from build123d import *

# Parameters (mm, degrees)
EXTRUDE_START          = 700
SKETCH_1_R             = 15
EXTRUDE_1_DEPTH        = 15
PATTERN_LINEAR_1_COUNT = 2
PATTERN_LINEAR_1_PITCH = 77
SKETCH_2_W             = 62
SKETCH_2_H             = 7
EXTRUDE_2_DEPTH        = 70
SKETCH_3_R             = 11
CUT_EXTRUDE_2_DEPTH    = 105
FILLET_1_R             = 5


with BuildPart() as part:
    # Sketch 1 → Extrude 1 (new body)
    with BuildSketch(Plane.XY.offset(-2290.827909759).offset(EXTRUDE_START)):
        with BuildLine():
            Line((4, 81), (-196, 81))
            ThreePointArc((-196, 81), (-230.605231181, 110.758056189), (-206.365638709, 149.429830005))
            Line((-206.365638709, 149.429830005), (-111, 179))
            Line((-111, 179), (17.209362926, 179))
            ThreePointArc((17.209362926, 179), (40.340952707, 173.32752592), (58.22400875, 157.597182169))
            Line((58.22400875, 157.597182169), (67.202929165, 144.719436434))
            ThreePointArc((67.202929165, 144.719436434), (67.865505184, 134.373682044), (59, 129))
            Line((59, 129), (4, 129))
            Line((4, 129), (4, 81))
        make_face()
        with Locations((-196, 116)):
            Circle(SKETCH_1_R, mode=Mode.SUBTRACT)
    extrude(amount=EXTRUDE_1_DEPTH)


with BuildPart() as pattern_linear_1_1:
    # Pattern Linear 1: pattern copy
    add(part.part.moved(Location(Vector(0, 0, 1) * (1 * PATTERN_LINEAR_1_PITCH))))


with BuildPart() as part_1:
    add(part.part)

    add(pattern_linear_1_1.part)  # Extrude 2 merges Pattern Linear 1_1
    # Sketch 2 → Extrude 2 (add)
    with BuildSketch(Plane.ZY.offset(-4)):
        with Locations((-1544.827909759, 120.5)):
            Rectangle(SKETCH_2_W, SKETCH_2_H)
    extrude(amount=EXTRUDE_2_DEPTH)

    # Sketch 3 → Cut-Extrude 2 (cut, symmetric)
    with BuildSketch(Plane(origin=(0, 0, -1513.827909759), x_dir=(-1, 0, 0), z_dir=(0, 0, -1))):
        with Locations(Location((80.605231181, 144, 0), (0, 0, 180))):
            Circle(SKETCH_3_R)
    extrude(amount=CUT_EXTRUDE_2_DEPTH, both=True, mode=Mode.SUBTRACT)

    # Fillet 1
    fillet_1_edges = [part_1.edges().sort_by_distance(p)[0] for p in [
        (4, 129, -1583.327909759),
        (4, 129, -1506.327909759),
    ]]
    fillet(fillet_1_edges, radius=FILLET_1_R)


solid = part_1.part
Can you work these out from the model? Positions are in its coordinate system, mm. A direction names the side the tool comes from. Coordinates: 2 decimals unless noted, no trailing zeros. Write each loop counter-clockwise with the first axis right and the second up, starting at its lowest first coordinate (ties: lowest second). Pieces come first, ordered by that corner, then holes.
Q1. Which directions (+Z, -Z, +X, -X, +Y, -Y) give clear straight access to the entire face, cutting with the end or side of a thin tool? Please do faces 4 (the face through (-31, 124, -1545)), 5 (the face through (-66, 121, -1545)), 6 (the face through (62.65, 151.25, -1583.43)), 7 (the face through (-31, 117, -1545)), 8 (the face through (34, 129, -1583)).
Results found:
face 4: +X, -X, +Y
face 5: -X, +Y, -Y
face 6: +Z, -Z, +X, +Y
face 7: +X, -X, -Y
face 8: +Z, -Z, +X, -Y
Q2. Imagine slicing it at B-B, the plane x = -6.5. List the corners of the cut face in (y, z) for me.
Results found:
outline: (81, -1590.83) - (179, -1590.83) - (179, -1575.83) - (124, -1575.83) - (124, -1513.83) - (179, -1513.83) - (179, -1498.83) - (81, -1498.83) - (81, -1513.83) - (117, -1513.83) - (117, -1575.83) - (81, -1575.83) - close
Q3. Imagine slicing it at D-D, the plane y = 90.5. List the corners of the cut face in (x, z) for me, plus the area to 3 significant figures.
Results found:
outline: (-219.97, -1590.83) - (4, -1590.83) - (4, -1575.83) - (-219.97, -1575.83) - close; (-219.97, -1513.83) - (4, -1513.83) - (4, -1498.83) - (-219.97, -1498.83) - close
area: 6,720 mm2
Q4. Imagine slicing it at C-C, the plane x = -137.5. List the corners of the cut face in (y, z) for me, plus the area to 3 significant figures.
Results found:
outline: (81, -1590.83) - (170.78, -1590.83) - (170.78, -1575.83) - (81, -1575.83) - close; (81, -1513.83) - (170.78, -1513.83) - (170.78, -1498.83) - (81, -1498.83) - close
area: 2,690 mm2
Q5. For P1, Ø7.5, axis at y = 120, z = -1554, coming from the -X side; P2, Ø4, axis at x = -71.5, z = -1517.5, coming from the +Y side; P3, Ø6, axis at x = -68.5, z = -1530, coming from the +Y side; P4, Ø7.5, axis at x = 38, z = -1584.5, coming from the -Y side, each with a flat end and sliding along its axis, tell me the tip position at first contact or that it passes through.
Results found:
P1: stops at x = -66
P2: passes through
P3: stops at y = 124
P4: stops at y = 129
Q6. If we mould it in two halves opening along Y, with no side actions, what happens to faces 1 (the face through (-82.037, 133.094, -1583.433)), 2 (the face through (5, 127, -1583)), 3 (the face through (-230.5, 110.1, -1583.4))? For each: +Y half, -Y half, draft (parallel to the pull), parting line (faces both ways), or undercut.
Results found:
face 1: undercut
face 2: -Y half
face 3: parting line
Q7. Please list where these lines run through material, in increasing order: L1, parallel to Z at x = -92, y = 142; L2, parallel to X at y = 144, z = -1505.25; L3, parallel to Y at x = -30, z = -1528.
Results found:
L1: z = -1590.83 to -1575.83, -1513.83 to -1498.83
L2: x = -217 to -91.61, -69.61 to 67.66
L3: y = 117 to 124
Q8. Imagine slicing it at A-A, the plane z = -1582.5. List the corners of the cut face in (x, y) for me, plus the area to 3 significant figures.
Results found:
outline: (-206.37, 149.43) arc R35 ccw to (-196, 81) - (4, 81) - (4, 124) arc R5 cw to (9, 129) - (59, 129) arc R10 ccw to (67.2, 144.72) - (58.22, 157.6) arc R50 ccw to (17.21, 179) - (-111, 179) - close; hole circle Ø30 at (-196, 116); hole circle Ø22 at (-80.61, 144)
area: 22,000 mm2
